Here's how the part is built. I have some questions about the finished solid (model axes, mm). A direction names the side the tool comes from. Round coordinates to 2 decimals unless told otherwise and drop trailing zeros. Write each loop counter-clockwise with the first axis right and the second up, starting at its lowest first coordinate (ties: lowest second). Pieces come first, ordered by that corner, then holes. Notation, with made-up numbers: (-1, 80) -> (57, 80) arc R20 ccw to (57, 115) -> close; hole circle Ø11 at (54.25, -24). An arc over 180 degrees is marked (long way). Put each result on its own line as item: value. Start each with the question number.
1) Which directions (+Z, -Z, +X, -X, +Y, -Y) give clear straight access to the entire face, cutting with the end or side of a thin tool? Please do faces 5 (the cylindrical face through (35.2, 7.6, -0.4)), 6 (the flat face through (30.1, 8, -2.4)), 7 (the flat face through (-34.85, 7, -1)).
2) I want a section at A-A, the plane x = 0. List the corners of the cut face in (y, z) for me.
3) I want a section at D-D, the plane z = 19. List the corners of the cut face in (x, y) for me, then the cut area to 3 significant figures.
4) I want a section at C-C, the plane y = 6. List the corners of the cut face in (x, z) for me.
5) We'd pull the mould along Z, two halves only. Please class faces 1 (the cylindrical face through (-35.2, 7.6, 0.4)), 2 (the cylindrical face through (13.6, 4.44, -32.79)), 3 (the flat face through (-1, 7, 34.85)), 4 (the flat face through (0, 7.56, -35)): released by +Z, released by -Z, zero draft, split by the parting line, or undercut.
6) I want a section at B-B, the plane z = 0. List the corners of the cut face in (x, y) for me, then the cut area to 3 significant figures.
7) Will these pins go through, and if not, where does the flat tip stop? P1, Ø3, axis at x = -14, y = 5.5, coming from the +Z side; P2, Ø4.5, axis at x = 0, y = 6, coming from the -Z side; P3, Ø2.5, axis at y = 6, z = 0, coming from the +X side; P4, Ø0.5, axis at x = -0.5, z = -34.5, coming from the -Y side.
8) If I drill on line 1 along Y through (x, z) = (-35, 0); line 2 along X through (y, z) = (8.6, 0); line 3 along X through (y, z) = (4, 31), over which ranges is the centre line in solid material (lowest first)? Write a range as [from, to].
from build123d import *

# Parameters (mm, degrees)
SKETCH2_W          = 7
SKETCH2_H          = 10
CUT_EXTRUDE1_DEPTH = 52.004901725
CUT_EXTRUDE2_START = 34.85
SKETCH3_R          = 1.65
CUT_EXTRUDE2_DEPTH = 10.65
CIRPATTERN1_COUNT  = 4
SKETCH4_R          = 1
CUT_EXTRUDE3_DEPTH = 52.004901895
CIRPATTERN3_COUNT  = 4


with BuildPart() as part:
    # Sketch1 → Revolve1 (revolve)
    with BuildSketch(Plane.XY, mode=Mode.PRIVATE) as revolve1_sk:
        Polygon((34, 0), (34, 8), (30, 8), (30, 9), (35.5, 9), (35.5, 0), align=None)
    revolve(revolve1_sk.sketch.rotate(Axis((0, -1.347881032, 0), (0, 1, 0)), 90), axis=Axis((0, -1.347881032, 0), (0, 1, 0)))

    # Sketch2 → Cut-Extrude1 (cut, through all)
    with BuildSketch(Plane.XY):
        with Locations((0, 2.56)):
            Rectangle(SKETCH2_W, SKETCH2_H)
    extrude(amount=-CUT_EXTRUDE1_DEPTH, mode=Mode.SUBTRACT)

    # Sketch3 → Cut-Extrude2 (cut)
    with BuildSketch(Plane.XY.offset(CUT_EXTRUDE2_START)):
        with Locations(Location((0, 6, 0), (0, 0, 180))):
            Circle(SKETCH3_R)
    cut_extrude2 = extrude(amount=CUT_EXTRUDE2_DEPTH, mode=Mode.SUBTRACT)

    # CirPattern1: Cut-Extrude2 ×4 about axis, 1 skipped
    cirpattern1_axis = Axis((0, 0, 0), (0, -1, 0))
    add([cut_extrude2.rotate(cirpattern1_axis, i * 360 / CIRPATTERN1_COUNT) for i in range(1, CIRPATTERN1_COUNT) if i not in (2,)], mode=Mode.SUBTRACT)

    # Sketch4 → Cut-Extrude3 (cut, through all)
    with BuildSketch(Plane.XY):
        with Locations(Location((0, 6, 0), (0, 0, 180))):
            Circle(SKETCH4_R)
    cut_extrude3 = extrude(amount=CUT_EXTRUDE3_DEPTH, mode=Mode.SUBTRACT)

    # CirPattern3: Cut-Extrude3 ×4 about axis, 1 skipped
    cirpattern3_axis = Axis((0, -1.347881032, 0), (0, -1, 0))
    add([cut_extrude3.rotate(cirpattern3_axis, i * 360 / CIRPATTERN3_COUNT) for i in range(1, CIRPATTERN3_COUNT) if i not in (2,)], mode=Mode.SUBTRACT)


solid = part.part
Findings:
1. face 5: +X
1. face 6: -Y
1. face 7: -X
2. outline: (0, 34) -> (5, 34) -> (5, 34.85) -> (4.35, 34.85) -> (4.35, 35.5) -> (0, 35.5) -> close; (7, 34) -> (8, 34) -> (8, 30) -> (9, 30) -> (9, 35.5) -> (7.65, 35.5) -> (7.65, 34.85) -> (7, 34.85) -> close; (7.56, -35.5) -> (9, -35.5) -> (9, -30) -> (8, -30) -> (8, -34) -> (7.56, -34) -> close
3. outline: (-29.99, 0) -> (-28.2, 0) -> (-28.2, 8) -> (-23.22, 8) -> (-23.22, 9) -> (-29.99, 9) -> close; (23.22, 8) -> (28.2, 8) -> (28.2, 0) -> (29.99, 0) -> (29.99, 9) -> (23.22, 9) -> close
3. area: 42.2 mm2
4. outline: (-35.46, -1.65) arc R35.5 ccw to (-3.5, -35.33) -> (-3.5, -33.82) arc R34 cw to (-33.99, -1) -> (-34.85, -1) -> (-34.85, -1.65) -> close; (-35.46, 1.65) -> (-34.85, 1.65) -> (-34.85, 1) -> (-33.99, 1) arc R34 cw to (-1, 33.99) -> (-1, 34.85) -> (-1.65, 34.85) -> (-1.65, 35.46) arc R35.5 ccw to start; (1, 33.99) arc R34 cw to (33.99, 1) -> (34.85, 1) -> (34.85, 1.65) -> (35.46, 1.65) arc R35.5 ccw to (1.65, 35.46) -> (1.65, 34.85) -> (1, 34.85) -> close; (3.5, -35.33) arc R35.5 ccw to (35.46, -1.65) -> (34.85, -1.65) -> (34.85, -1) -> (33.99, -1) arc R34 cw to (3.5, -33.82) -> close
5. face 1: undercut
5. face 2: split by the parting line
5. face 3: released by +Z
5. face 4: zero draft
6. outline: (-35.5, 0) -> (-34, 0) -> (-34, 5) -> (-34.85, 5) -> (-34.85, 4.35) -> (-35.5, 4.35) -> close; (-35.5, 7.65) -> (-34.85, 7.65) -> (-34.85, 7) -> (-34, 7) -> (-34, 8) -> (-30, 8) -> (-30, 9) -> (-35.5, 9) -> close; (30, 8) -> (34, 8) -> (34, 7) -> (34.85, 7) -> (34.85, 7.65) -> (35.5, 7.65) -> (35.5, 9) -> (30, 9) -> close; (34, 0) -> (35.5, 0) -> (35.5, 4.35) -> (34.85, 4.35) -> (34.85, 5) -> (34, 5) -> close
6. area: 27.3 mm2
7. P1: stops at z = 33.23
7. P2: stops at z = -35.5
7. P3: stops at x = 34.85
7. P4: stops at y = 7.56
8. line 1: y = [0, 4.35], [7.65, 9]
8. line 2: x = [-35.5, -30], [30, 35.5]
8. line 3: x = [-17.3, -13.96], [13.96, 17.3]
